The listing builds one solid part. Answer for the finished solid, in the listing's coordinates (mm). Round coordinates to 2 decimals unless told otherwise and drop trailing zeros. Write each loop counter-clockwise with the first axis right and the second up, starting at its lowest first coordinate (ties: lowest second). Pieces come first, ordered by that corner, then holes. Notation, with made-up numbers: (84.25, 35) - (91.25, 35) arc R12 cw to (91.25, 53) - close; hole circle Ø3 at (43, 81). An arc over 180 degrees is marked (long way). Use a Markdown table: item, result. Add a question column.
1) A cutting plane is placed at A-A (y = 78.5). Give the vertices of the cut face in (x, z), then the cut area to 3 significant figures.
2) Find the intervals of material crossed by probe 1 along Z at (x, y) = (0, -137.75); probe 2 along X at (y, z) = (-135, 26); probe 3 along Y at (x, z) = (0, 17), in increasing order. Write a range as from..to.
3) Each of these flat-tipped pins is pushed along its axis until it touches: P1, Ø2.5, axis at x = 0, y = 55, coming from the -Z side; P2, Ø3, axis at x = 0, y = -55, coming from the -Z side. Where does it stop, or does it pass through?
4) Determine the mould class of faces 1 (the flat face through (0, 2, 30)), 2 (the cylindrical face through (-0.1, 78.6, 13.5)), 3 (the flat face through (-5, -2, 0)), 4 (the flat face through (0, 2, -30)) for opening direction Z: +Z half, -Z half, draft (parallel to the pull), parting line (faces both ways), or undercut.
```python
from build123d import *

# Parameters (mm, degrees)
SKETCH1_W                  = 10
SKETCH1_H                  = 293
BOSS_EXTRUDE1_DEPTH        = 30
M4_TAPPED_HOLE1_AT_2_COUNT = 2
M4_TAPPED_HOLE1_AT_2_PITCH = 270
M4_TAPPED_HOLE1_AT_3_COUNT = 2
M4_TAPPED_HOLE1_AT_3_PITCH = 80
M4_TAPPED_HOLE1_AT_4_COUNT = 2
M4_TAPPED_HOLE1_AT_4_PITCH = 190
M6_TAPPED_HOLE1_D          = 5


with BuildPart() as part:
    # Sketch1 → Boss-Extrude1 (new, symmetric)
    with BuildSketch(Plane.XY):
        Rectangle(SKETCH1_W, SKETCH1_H)
    extrude(amount=BOSS_EXTRUDE1_DEPTH, both=True)

    # Sketch4 → M4 Tapped Hole1 (revolve, cut)
    with BuildSketch(Plane(origin=(0, 135, 30), x_dir=(0, -1, 0), z_dir=(1, 0, 0))):
        Polygon((0, 0), (0, 12.491420021), (1.65, 11.5), (1.65, 0), align=None)
    m4_tapped_hole1 = revolve(axis=Axis((0, 135, 36.35), (0, 0, -1)), mode=Mode.SUBTRACT)

    # M4 Tapped Hole1 at 2: M4 Tapped Hole1 ×2
    with Locations(*[(0, -i * M4_TAPPED_HOLE1_AT_2_PITCH, 0) for i in range(1, M4_TAPPED_HOLE1_AT_2_COUNT)]):
        add(m4_tapped_hole1, mode=Mode.SUBTRACT)

    # M4 Tapped Hole1 at 3: M4 Tapped Hole1 ×2
    with Locations(*[(0, -i * M4_TAPPED_HOLE1_AT_3_PITCH, 0) for i in range(1, M4_TAPPED_HOLE1_AT_3_COUNT)]):
        add(m4_tapped_hole1, mode=Mode.SUBTRACT)

    # M4 Tapped Hole1 at 4: M4 Tapped Hole1 ×2
    with Locations(*[(0, -i * M4_TAPPED_HOLE1_AT_4_PITCH, 0) for i in range(1, M4_TAPPED_HOLE1_AT_4_COUNT)]):
        add(m4_tapped_hole1, mode=Mode.SUBTRACT)

    # Sketch6 → M4 Tapped Hole2 (revolve, cut)
    with BuildSketch(Plane(origin=(0, -146.5, 0), x_dir=(0, 0, -1), z_dir=(1, 0, 0))):
        Polygon((0, 0), (0, 12.491420021), (1.65, 11.5), (1.65, 0), align=None)
    m4_tapped_hole2 = revolve(axis=Axis((0, -152.85, 0), (0, 1, 0)), mode=Mode.SUBTRACT)

    # Mirror1: M4 Tapped Hole2 across plane
    add(m4_tapped_hole2.mirror(Plane.ZX), mode=Mode.SUBTRACT)

    # M6 Tapped Hole1 (through all)
    with Locations(Plane(origin=(5, 0, 0), x_dir=(0, 0, -1), z_dir=(1, 0, 0))):
        with Locations((-16, 78.5), (16, 78.5), (16, 108.5), (-16, 108.5)):
            Hole(M6_TAPPED_HOLE1_D / 2)

    # Mirror2: M4 Tapped Hole1 across plane
    add(m4_tapped_hole1.mirror(Plane.XY), mode=Mode.SUBTRACT)

    # Mirror2 copy 1 sketch → Mirror2 copy 1 (revolve, cut)
    with BuildSketch(Plane(origin=(0, -135, -30), x_dir=(0, -1, 0), z_dir=(1, 0, 0))):
        Polygon((0, 0), (0, -12.491420021), (1.65, -11.5), (1.65, 0), align=None)
    revolve(axis=Axis((0, -135, -36.35), (0, 0, -1)), mode=Mode.SUBTRACT)

    # Mirror2 copy 2 sketch → Mirror2 copy 2 (revolve, cut)
    with BuildSketch(Plane(origin=(0, 55, -30), x_dir=(0, -1, 0), z_dir=(1, 0, 0))):
        Polygon((0, 0), (0, -12.491420021), (1.65, -11.5), (1.65, 0), align=None)
    revolve(axis=Axis((0, 55, -36.35), (0, 0, -1)), mode=Mode.SUBTRACT)

    # Mirror2 copy 3 sketch → Mirror2 copy 3 (revolve, cut)
    with BuildSketch(Plane(origin=(0, -55, -30), x_dir=(0, -1, 0), z_dir=(1, 0, 0))):
        Polygon((0, 0), (0, -12.491420021), (1.65, -11.5), (1.65, 0), align=None)
    revolve(axis=Axis((0, -55, -36.35), (0, 0, -1)), mode=Mode.SUBTRACT)


solid = part.part
```
Entries:
| question | item | result |
|---|---|---|
| 1 | outline | (-5, -30) - (5, -30) - (5, -18.5) - (-5, -18.5) - close; (-5, -13.5) - (5, -13.5) - (5, 13.5) - (-5, 13.5) - close; (-5, 18.5) - (5, 18.5) - (5, 30) - (-5, 30) - close |
| 1 | area | 500 mm² |
| 2 | probe 1 | z = -30..-1.65, 1.65..30 |
| 2 | probe 2 | x = -5..-1.65, 1.65..5 |
| 2 | probe 3 | y = -146.5..76.21, 80.79..106.21, 110.79..146.5 |
| 3 | P1 | stops at z = -18.26 |
| 3 | P2 | stops at z = -18.41 |
| 4 | face 1 | +Z half |
| 4 | face 2 | undercut |
| 4 | face 3 | draft |
| 4 | face 4 | -Z half |
